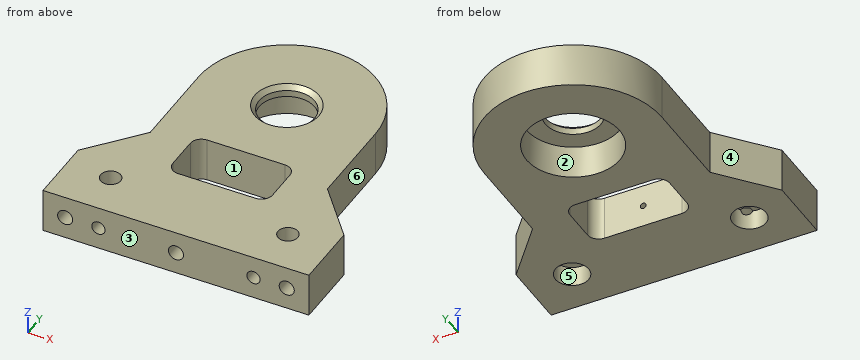
```python
from build123d import *

# Parameters (mm, degrees)
SKETCH_1_R                = 12.5
EXTRUDE_1_DEPTH           = 10
HOLE_WIZARD_M8_1_D        = 6.8
HOLE_WIZARD_M8_1_DEPTH    = 33.75
HOLE_WIZARD_M8_1_TIP      = 2.042926105
HOLE_WIZARD_6_0_6_1_D     = 6
HOLE_WIZARD_6_0_6_1_DEPTH = 15
HOLE_WIZARD_6_0_6_1_TIP   = 1.802581857
SKETCH_6_R                = 21
CUT_EXTRUDE_1_DEPTH       = 15
CHAMFER_1_SIZE            = 2
HOLE_WIZARD_2_D           = 9
HOLE_WIZARD_2_CBORE_D     = 15
HOLE_WIZARD_2_CBORE_DEPTH = 9
CUT_EXTRUDE_2_DEPTH       = 150.080515159


with BuildPart() as part:
    # 草图1 → 凸台-拉伸1 (new, symmetric)
    with BuildSketch(Plane.XY):
        with BuildLine():
            Line((-60, 30), (-40, 53.835071852))
            Line((-40, 53.835071852), (-40, 95))
            ThreePointArc((-40, 95), (0, 135), (40, 95))
            Line((40, 95), (40, 53.835071852))
            Line((40, 53.835071852), (60, 30))
            Line((60, 30), (60, 0))
            Line((60, 0), (-60, 0))
            Line((-60, 0), (-60, 30))
        make_face()
        with Locations((0, 95)):
            Circle(SKETCH_1_R, mode=Mode.SUBTRACT)
    extrude(amount=EXTRUDE_1_DEPTH, both=True)

    # M8 螺纹孔1
    with Locations(Plane(origin=(0, 0, 0), x_dir=(-1, 0, 0), z_dir=(0, -1, 0))):
        with Locations((50, 0), (0, 0), (-50, 0)):
            Hole(HOLE_WIZARD_M8_1_D / 2, depth=HOLE_WIZARD_M8_1_DEPTH)
            with Locations((0, 0, -(HOLE_WIZARD_M8_1_DEPTH + HOLE_WIZARD_M8_1_TIP / 2))):  # 118° drill point
                Cone(0, HOLE_WIZARD_M8_1_D / 2, HOLE_WIZARD_M8_1_TIP, mode=Mode.SUBTRACT)

    # Ø6.0 (6) 直径孔1
    with Locations(Plane(origin=(0, 0, 0), x_dir=(-1, 0, 0), z_dir=(0, -1, 0))):
        with Locations((-35, 0), (35, 0)):
            Hole(HOLE_WIZARD_6_0_6_1_D / 2, depth=HOLE_WIZARD_6_0_6_1_DEPTH)
            with Locations((0, 0, -(HOLE_WIZARD_6_0_6_1_DEPTH + HOLE_WIZARD_6_0_6_1_TIP / 2))):  # 118° drill point
                Cone(0, HOLE_WIZARD_6_0_6_1_D / 2, HOLE_WIZARD_6_0_6_1_TIP, mode=Mode.SUBTRACT)

    # 草图6 → 切除-拉伸1 (cut)
    with BuildSketch(Plane.XY.offset(-10)):
        with Locations((0, 95)):
            Circle(SKETCH_6_R)
    extrude(amount=CUT_EXTRUDE_1_DEPTH, mode=Mode.SUBTRACT)

    # 倒角1
    chamfer_1_edges = [part.edges().sort_by_distance(p)[0] for p in [
        (-12.5, 95, 10),
    ]]
    chamfer(chamfer_1_edges, length=CHAMFER_1_SIZE)

    # 打孔尺寸(%根据)内六角圆柱头螺钉的类型2 (through all)
    with Locations(Plane(origin=(0, 0, -10), x_dir=(-1, 0, 0), z_dir=(0, 0, -1))):
        with Locations((-40, 20), (40, 20)):
            CounterBoreHole(HOLE_WIZARD_2_D / 2, HOLE_WIZARD_2_CBORE_D / 2, HOLE_WIZARD_2_CBORE_DEPTH)

    # 草图13 → 切除-拉伸2 (cut, through all)
    with BuildSketch(Plane(origin=(0, 0, -10), x_dir=(-1, 0, 0), z_dir=(0, 0, -1))):
        with BuildLine():
            Line((17.5, 60), (-17.5, 60))
            ThreePointArc((-17.5, 60), (-21.035533906, 58.535533906), (-22.5, 55))
            Line((-22.5, 55), (-22.5, 40))
            ThreePointArc((-22.5, 40), (-21.035533906, 36.464466094), (-17.5, 35))
            Line((-17.5, 35), (17.5, 35))
            ThreePointArc((17.5, 35), (21.035533906, 36.464466094), (22.5, 40))
            Line((22.5, 40), (22.5, 55))
            ThreePointArc((22.5, 55), (21.035533906, 58.535533906), (17.5, 60))
        make_face()
    extrude(amount=-CUT_EXTRUDE_2_DEPTH, mode=Mode.SUBTRACT)


solid = part.part
```
Build history of the part. All positions in model axes, mm. Face numbers are marked on the shaded views. A direction names the side the tool comes from. Give positions to 0.01 mm unless a question says otherwise; leave off trailing zeros. Loops run counter-clockwise (first coordinate to the right, second up) from the corner with the lowest first, then second, coordinate; pieces in that order, holes last. Notation, with made-up numbers: (20.5, 64.25) -> (75.5, 64.25) arc R16 ccw to (75.5, 68.25) -> close; hole circle Ø5 at (-1, 36.25). An arc over 180 degrees is marked (long way). One line per question, with ' | ' between items. Start each with the question number.
1) Cut at A-A (z = -6). Give the cut face in (x, y), plus the area to 3 significant figures.
2) 3-axis set-ups, long thin cutter, end or side, ignore diameter. For the marked faces 1, 2 and 3: which of +Z, -Z, +X, -X, +Y, -Y reach the whole face in a straight line?
3) Cut at B-B (y = 20). Give the cut face in (x, z), plus the area to 3 significant figures.
4) Pin check, flat tips, straight feed: pin 1 (3 mm diameter, centred on y = 33.5, z = -7, fed in from +X); pin 2 (8 mm diameter, centred on x = -50, z = 0, fed in from +Y); pin 3 (21 mm diameter, centred on x = 4, y = 102, fed in from -Z). Stop position of each tip, or through.
5) Two-plate mould, pull along X, no slides. Class the marked faces 4, 5 and 6: released by +X, released by -X, zero draft, split by the parting line, or undercut.
6) Probe L1, parallel to Y at x = 0, z = -8; L2, parallel to X at y = 20, z = -6.25; L3, parallel to Y at x = -5.5, z = -3.25. List the from-to ranges inside material, lowest first.
Return value:
1) outline: (-60, 0) -> (60, 0) -> (60, 30) -> (40, 53.84) -> (40, 95) arc R40 ccw to (-40, 95) -> (-40, 53.84) -> (-60, 30) -> close; hole circle Ø15 at (-40, 20); hole (-22.5, 40) arc R5 ccw to (-17.5, 35) -> (17.5, 35) arc R5 ccw to (22.5, 40) -> (22.5, 55) arc R5 ccw to (17.5, 60) -> (-17.5, 60) arc R5 ccw to (-22.5, 55) -> close; hole circle Ø42 at (0, 95); hole circle Ø15 at (40, 20) | area: 8,950 mm^2
2) face 1: +Z, -Z | face 2: -Z | face 3: +Z, -Z, +X, -X, -Y
3) outline: (-60, -10) -> (-47.5, -10) -> (-47.5, -2.3) arc R3.4 cw (long way) to (-46.75, -1) -> (-44.5, -1) -> (-44.5, 10) -> (-60, 10) -> close; (-35.5, -1) -> (-32.5, -1) -> (-32.5, -10) -> (32.5, -10) -> (32.5, -1) -> (35.5, -1) -> (35.5, 10) -> (-35.5, 10) -> close; (44.5, -1) -> (46.75, -1) arc R3.4 cw (long way) to (47.5, -2.3) -> (47.5, -10) -> (60, -10) -> (60, 10) -> (44.5, 10) -> close; hole circle Ø6.8 at (0, 0) | area: 1,820 mm^2
4) pin 1: x = 58.32 | pin 2: y = 46.68 | pin 3: z = 5
5) face 4: released by -X | face 5: undercut | face 6: released by +X
6) L1: 0 to 35, 60 to 74, 116 to 135 | L2: -60 to -47.5, -32.5 to 32.5, 47.5 to 60 | L3: 0 to 35, 60 to 74.73, 115.27 to 134.62
